Geometry check sheet. Reference: the model listing, model coordinates, mm. Give positions to 0.01 mm unless a question says otherwise; leave off trailing zeros. Write each loop counter-clockwise with the first axis right and the second up, starting at its lowest first coordinate (ties: lowest second). Pieces come first, ordered by that corner, then holes. Notation, with made-up numbers: (85, -24) - (112, -24) arc R26 cw to (112, -9) - close; hole circle Ø4 at (18.25, 66). An arc over 180 degrees is marked (long way). Write item = value, one per line. Start each with the question number.
(1) Section check C-C, the plane z = -0.65. Enter the section's corners in (x, y).
(2) Depth check by flat-ended pin: pin 1 Ø0.9 at (x, y) = (3.25, -3.93) entering from -Z. Enter the tip coordinate at first touch or a pass-through.
(3) Thickness scan on L1, parallel to Y at x = -3, z = -0.5; L2, parallel to Y at x = 3.25, z = -0.55; L3, parallel to X at y = 2, z = -0.2. Record the ranges inside material, lowest first.
(4) Section check A-A, the plane y = 0. Enter the section's corners in (x, z).
(5) Section check B-B, the plane x = -3.5. Enter the section's corners in (y, z), plus the area to 3 significant figures.
(6) Section check D-D, the plane x = 2.75. Enter the section's corners in (y, z), plus the area to 3 significant figures.
```python
from build123d import *

# Parameters (mm, degrees)
SKETCH1_R  = 0.75
BODY_DEPTH = 0.8


with BuildPart() as part:
    # Sketch1 → Body (new body)
    with BuildSketch(Plane.XY):
        with BuildLine():
            Line((1.865360941, -4.503379682), (2.48744231, -6.005216961))
            ThreePointArc((2.48744231, -6.005216961), (0, 6.5), (-2.48744231, -6.005216961))
            Line((-2.48744231, -6.005216961), (-1.865360941, -4.503379682))
            ThreePointArc((-1.865360941, -4.503379682), (-2.152695679, -2.907918451), (-3.723088598, -2.5055208))
            ThreePointArc((-3.723088598, -2.5055208), (-4.504717999, -2.440543041), (-4.999049926, -1.831607432))
            ThreePointArc((-4.999049926, -1.831607432), (0, 4.8), (4.999049926, -1.831607432))
            ThreePointArc((4.999049926, -1.831607432), (4.504717999, -2.440543041), (3.723088598, -2.5055208))
            ThreePointArc((3.723088598, -2.5055208), (2.152695679, -2.907918451), (1.865360941, -4.503379682))
        make_face()
        with Locations(Location((3.25118024, -3.929354533, 0), (0, 0, 180))):
            Circle(SKETCH1_R, mode=Mode.SUBTRACT)
        with Locations((-3.25118024, -3.929354533)):
            Circle(SKETCH1_R, mode=Mode.SUBTRACT)
    extrude(amount=-BODY_DEPTH)


solid = part.part
```
Model answer:
q1.outline = (-5, -1.83) arc R5.2 cw (long way) to (5, -1.83) arc R1 cw to (3.72, -2.51) arc R1.5 ccw to (1.87, -4.5) - (2.49, -6.01) arc R6.5 ccw (long way) to (-2.49, -6.01) - (-1.87, -4.5) arc R1.5 ccw to (-3.72, -2.51) arc R1 cw to start; hole circle Ø1.5 at (-3.25, -3.93); hole circle Ø1.5 at (3.25, -3.93)
q2.pin_1 = through
q3.L1 = -5.77 to -4.64, -3.22 to -2.45, 3.85 to 5.77
q3.L2 = -5.63 to -4.68, -3.18 to -2.43, 3.66 to 5.63
q3.L3 = -6.18 to -4.61, 4.61 to 6.18
q4.outline = (-6.5, -0.8) - (-5.18, -0.8) - (-5.18, 0) - (-6.5, 0) - close; (5.18, -0.8) - (6.5, -0.8) - (6.5, 0) - (5.18, 0) - close
q5.outline = (-5.48, -0.8) - (-4.64, -0.8) - (-4.64, 0) - (-5.48, 0) - close; (-3.22, -0.8) - (-2.45, -0.8) - (-2.45, 0) - (-3.22, 0) - close; (3.45, -0.8) - (5.48, -0.8) - (5.48, 0) - (3.45, 0) - close
q5.area = 2.91 mm²
q6.outline = (-5.89, -0.8) - (-4.49, -0.8) - (-4.49, 0) - (-5.89, 0) - close; (-3.37, -0.8) - (-2.52, -0.8) - (-2.52, 0) - (-3.37, 0) - close; (4.01, -0.8) - (5.89, -0.8) - (5.89, 0) - (4.01, 0) - close
q6.area = 3.31 mm²
